CAD build for the part. Positions are in the model's coordinates, mm. A direction names the side the tool comes from. Give positions to 0.01 mm unless a question says otherwise; leave off trailing zeros. Write each loop counter-clockwise with the first axis right and the second up, starting at its lowest first coordinate (ties: lowest second). Pieces come first, ordered by that corner, then holes. Notation, with made-up numbers: (-38.75, 33.5) - (-19.75, 33.5) arc R14 cw to (-19.75, 47.5) - close; hole circle Ø2 at (-40, 76.5). An arc over 180 degrees is marked (long way). Answer as a JSON object with one key per item and string values.
from build123d import *

# Parameters (mm, degrees)
SKETCH1_R           = 2.5
SKETCH3_R           = 32.5
BOSS_EXTRUDE1_DEPTH = 6
SKETCH5_R           = 4.5
CUT_EXTRUDE1_DEPTH  = 6
CIRPATTERN1_COUNT   = 6
SKETCH6_R           = 5
BOSS_EXTRUDE2_DEPTH = 45
SKETCH7_R           = 10
BOSS_EXTRUDE3_DEPTH = 8
CHAMFER1_SIZE       = 1.5
CUT_EXTRUDE2_START  = -8
CUT_EXTRUDE2_DEPTH  = 8
FILLET1_R           = 2
SKETCH9_R           = 57.5
SKETCH9_R_2         = 35
CUT_EXTRUDE3_DEPTH  = 323.720467373


with BuildPart() as part:
    # Sweep1: sweep along a path in Sketch2
    with BuildLine(Plane(origin=(0, 0, 0), x_dir=(1, 0, 0), z_dir=(0, 1, 0))) as sweep1_path:
        Line((0, 0), (282.5, 0))
        ThreePointArc((282.5, 0), (297.5, 15), (282.5, 30))
        Line((282.5, 30), (0, 30))
    # Sketch1 → Sweep1 (sweep)
    with BuildSketch(Plane(origin=(0, 0, 0), x_dir=(0, 0, -1), z_dir=(1, 0, 0))):
        Circle(SKETCH1_R)
    sweep1 = sweep(path=sweep1_path.line)

    # Sketch3 → Boss-Extrude1 (add)
    with BuildSketch(Plane.ZY):
        with Locations((-15, -15)):
            Circle(SKETCH3_R)
    extrude(amount=-BOSS_EXTRUDE1_DEPTH)

    # Mirror3: Sweep1 across plane
    add(sweep1.mirror(Plane.ZX.offset(-15)))

    # Sketch4 → Revolve1 (revolve)
    with BuildSketch(Plane(origin=(0, -15, 0), x_dir=(-1, 0, 0), z_dir=(0, 1, 0))):
        Polygon((0, -15), (0, 42.5), (6, 42.5), (6, 17.5), (76, 17.5), (76, -5), (78, -5), (78, -15), align=None)
    revolve(axis=Axis((-78, -15, -15), (1, 0, 0)))

    # Sketch5 → Cut-Extrude1 (cut)
    with BuildSketch(Plane.ZY.offset(6)):
        with Locations((-15, 32)):
            Circle(SKETCH5_R)
    cut_extrude1 = extrude(amount=-CUT_EXTRUDE1_DEPTH, mode=Mode.SUBTRACT)

    # CirPattern1: Cut-Extrude1 ×6 about axis
    cirpattern1_axis = Axis((0, -15, -15), (1, 0, 0))
    for i in range(1, CIRPATTERN1_COUNT):
        add(cut_extrude1.rotate(cirpattern1_axis, i * 360 / CIRPATTERN1_COUNT), mode=Mode.SUBTRACT)

    # Sketch6 → Boss-Extrude2 (add)
    with BuildSketch(Plane(origin=(0, -15, 0), x_dir=(-1, 0, 0), z_dir=(0, 1, 0))):
        with Locations(Location((56, -15, 0), (0, 0, 90))):
            Circle(SKETCH6_R)
    extrude(amount=-BOSS_EXTRUDE2_DEPTH)

    # Sketch7 → Boss-Extrude3 (add)
    with BuildSketch(Plane.XZ.offset(60)):
        with Locations(Location((-56, -15, 0), (0, 0, 270))):
            Circle(SKETCH7_R)
    extrude(amount=BOSS_EXTRUDE3_DEPTH)

    # Chamfer1
    chamfer1_edges = [part.edges().sort_by_distance(p)[0] for p in [
        (-56, -60, -5),
        (-56, -68, -5),
    ]]
    chamfer(chamfer1_edges, length=CHAMFER1_SIZE)

    # Sketch8 → Cut-Extrude2 (cut)
    with BuildSketch(Plane.XZ.offset(68).offset(CUT_EXTRUDE2_START)):
        with BuildLine():
            Line((-64.660254038, -20), (-64.660254038, -10))
            ThreePointArc((-64.660254038, -10), (-66, -15), (-64.660254038, -20))
        make_face()
        with BuildLine():
            Line((-64.660254038, -10), (-56, -5))
            ThreePointArc((-56, -5), (-61, -6.339745962), (-64.660254038, -10))
        make_face()
        with BuildLine():
            ThreePointArc((-47.339745962, -10), (-51, -6.339745962), (-56, -5))
            Line((-56, -5), (-47.339745962, -10))
        make_face()
        with BuildLine():
            ThreePointArc((-46, -15), (-46.340741737, -12.411809549), (-47.339745962, -10))
            Line((-47.339745962, -10), (-47.339745962, -20))
            ThreePointArc((-47.339745962, -20), (-46.340741737, -17.588190451), (-46, -15))
        make_face()
        with BuildLine():
            ThreePointArc((-56, -25), (-51, -23.660254038), (-47.339745962, -20))
            Line((-47.339745962, -20), (-56, -25))
        make_face()
        with BuildLine():
            Line((-56, -25), (-64.660254038, -20))
            ThreePointArc((-64.660254038, -20), (-61, -23.660254038), (-56, -25))
        make_face()
    extrude(amount=CUT_EXTRUDE2_DEPTH, mode=Mode.SUBTRACT)

    # Fillet1
    fillet1_edges = [part.edges().sort_by_distance(p)[0] for p in [
        (-76, -15, -47.5),
    ]]
    fillet(fillet1_edges, radius=FILLET1_R)

    # Sketch9 → Cut-Extrude3 (cut, through all)
    with BuildSketch(Plane.ZY.offset(6)):
        with Locations((-15, -15)):
            Circle(SKETCH9_R)
        with Locations((-15, -15)):
            Circle(SKETCH9_R_2, mode=Mode.SUBTRACT)
    extrude(amount=-CUT_EXTRUDE3_DEPTH, mode=Mode.SUBTRACT)


solid = part.part
(1) Probe L1, parallel to Y at x = 219.5, z = -30; L2, parallel to X at y = -42, z = -11.5; L3, parallel to X at y = -31, z = -22. List the from-to ranges inside material, lowest first. Write a range as [from, to].
Answer key:
{"L1": "y = [-32.5, -27.5], [-2.5, 2.5]", "L2": "x = [-76, 6]", "L3": "x = [-76, 6], [293.11, 298.31]"}
(2) Saw through at B-B, the plane y = -15. Give the cut face in (x, z).
Answer key:
{"outline": "(-78, -25) - (-76, -25) - (-76, -45.5) arc R2 ccw to (-74, -47.5) - (-6, -47.5) - (-6, -50) - (0, -50) - (0, -47.5) - (6, -47.5) - (6, 17.5) - (0, 17.5) - (0, 20) - (-6, 20) - (-6, 17.5) - (-74, 17.5) arc R2 ccw to (-76, 15.5) - (-76, -5) - (-78, -5) - close"}
(3) Pull direction Y, two halves, no side cores. Call faces 1 (the face through (-77.01, -18, -5.46)), 2 (the face through (-78, -15, -15)), 3 (the face through (-51.043, -53.466, -15.651)), 4 (the face through (-56, -68, -15)): pulls with the +Y half, pulls with the -Y half, needs draft (parallel to the pull), parting line crosses it, or undercut.
Answer key:
{"face 1": "parting line crosses it", "face 2": "needs draft", "face 3": "undercut", "face 4": "pulls with the -Y half"}
(4) Saw through at A-A, the plane z = -15. State how many separate pieces and enclosed holes the cut face has, and give its area (3 significant figures).
Answer key:
{"separate pieces": "3", "enclosed holes": "0", "area": "5,700 mm²"}
(5) 3-axis set-ups, long thin cutter, end or side, ignore diameter. For faces 5 (the face through (-60.27, -63.946, -22.535)), 6 (the face through (-51.73, -63.946, -7.465)), 7 (the face through (-64.66, -64, -15)), 8 (the face through (-47.34, -64, -15)): which of +Z, -Z, +X, -X, +Y, -Y reach the whole face in a straight line?
Answer key:
{"face 5": "-Z, -X, -Y", "face 6": "+Z, +X, -Y", "face 7": "+Z, -Z, -X, -Y", "face 8": "+Z, -Z, +X, -Y"}
(6) Flat gauge pins, fed straight in: P1, Ø4, axis at y = -43, z = -13.5, coming from the +X side; P2, Ø2.5, axis at y = -62.5, z = -17, coming from the +X side; P3, Ø21, axis at y = -25, z = -25, coming from the -X side; P4, Ø3, axis at y = -41.5, z = 4, coming from the -X side. Where does each tip first touch, or does it go through?
Answer key:
{"P1": "stops at x = 6", "P2": "stops at x = -47.34", "P3": "stops at x = -78", "P4": "stops at x = -75.91"}
(7) Saw through at C-C, the plane x = 52. Give the cut face in (y, z), and give its area (3 significant figures).
Answer key:
{"outline": "circle Ø5 at (-30, -30); circle Ø5 at (-30, 0); circle Ø5 at (0, -30); circle Ø5 at (0, 0)", "area": "78.5 mm²"}
